Part model, mm, in its own coordinate system. Coordinates: 2 decimals unless noted, no trailing zeros. Write each loop counter-clockwise with the first axis right and the second up, starting at its lowest first coordinate (ties: lowest second). Pieces come first, ordered by that corner, then holes. Notation, with made-up numbers: M 87.25,11.5 L 142.25,11.5 A24 cw 142.25,48.5 Z; hole C 85,-15 d10. An arc over 180 degrees is marked long. Use a Markdown table: item, result. Add a question column.
Q1. Slice it at A-A on z = 0. Write the cut outline in (x, y), then the cut area to 3 significant figures.
Q2. Slice it at C-C on x = -112. Write the cut outline in (y, z).
Q3. Wall check: L1, parallel to X at y = 50.5, z = 0; L2, parallel to Y at x = -55, z = 2.25; L3, parallel to Y at x = -97, z = 5. Give the ranges that are in metal, low to high. Write a range as from..to.
Q4. Pin check, flat tips, straight feed: pin 1 Ø1 at (y, z) = (90, -3) entering from -X; pin 2 Ø5 at (x, z) = (-106.5, -1.5) entering from -Y; pin 3 Ø6 at (x, z) = (-109.5, -4) entering from -Y; pin 4 Ø7.5 at (y, z) = (-0.5, 3.5) entering from +X. Stop position of each tip, or through.
Q5. Mould opens along X. For faces 1 (the flat face through (0, 0, 0)), 2 (the flat face through (-50, 0, 0)) say: released by +X, released by -X, zero draft, split by the parting line, or undercut.
Q6. Slice it at B-B on y = 71. Write the cut outline in (x, z).
from build123d import *

# Parameters (mm, degrees)
SKETCH2_R = 7.5


with BuildPart() as part:
    # Sweep1: sweep along a path in Sketch1
    with BuildLine(Plane.XY) as sweep1_path:
        Line((0, 0), (70, 0))
        ThreePointArc((70, 0), (91.213203436, 8.786796564), (100, 30))
        Line((100, 30), (100, 120))
        ThreePointArc((100, 120), (91.213203436, 141.213203436), (70, 150))
        Line((70, 150), (-120, 150))
        ThreePointArc((-120, 150), (-141.213203436, 141.213203436), (-150, 120))
        Line((-150, 120), (-150, 30))
        ThreePointArc((-150, 30), (-141.213203436, 8.786796564), (-120, 0))
        Line((-120, 0), (-50, 0))
    # Sketch2 → Sweep1 (sweep)
    with BuildSketch(Plane(origin=(0, 0, 0), x_dir=(0, 0, -1), z_dir=(1, 0, 0))):
        Circle(SKETCH2_R)
    sweep(path=sweep1_path.line)


solid = part.part
Recorded:
| question | item | result |
|---|---|---|
| 1 | outline | M -157.5,30 A37.5 ccw -120,-7.5 L -50,-7.5 L -50,7.5 L -120,7.5 A22.5 cw -142.5,30 L -142.5,120 A22.5 cw -120,142.5 L 70,142.5 A22.5 cw 92.5,120 L 92.5,30 A22.5 cw 70,7.5 L 0,7.5 L 0,-7.5 L 70,-7.5 A37.5 ccw 107.5,30 L 107.5,120 A37.5 ccw 70,157.5 L -120,157.5 A37.5 ccw -157.5,120 Z |
| 1 | area | 10,500 mm² |
| 2 | outline | C 0,0 d15; C 150,0 d15 |
| 3 | L1 | -157.5..-142.5, 92.5..107.5 |
| 3 | L2 | -7.15..7.15, 142.85..157.15 |
| 3 | L3 | -5.59..5.59, 144.41..155.59 |
| 4 | pin 1 | x = -157.07 |
| 4 | pin 2 | y = -7.5 |
| 4 | pin 3 | y = -7.43 |
| 4 | pin 4 | x = 95.57 |
| 5 | face 1 | undercut |
| 5 | face 2 | undercut |
| 6 | outline | C -150,0 d15; C 100,0 d15 |
